Can you work these out from the model? Positions are in its coordinate system, mm. Face numbers are marked on the shaded views. A direction names the side the tool comes from. Give positions to 0.01 mm unless a question says otherwise; leave off trailing zeros. Order: outer loops, then holes, each group sorted by start corner. A loop starts at its lowest first (then second) coordinate and runs counter-clockwise, first axis right, second up. Notation, with made-up numbers: M 24.25,-38 L 63.25,-38 A21 cw 63.25,-20 Z; hole C 85.25,64 d8. An arc over 180 degrees is marked long. Use one line per item in the form item = value. Start each with the question number.
1. I need wall thicknesses on L1, parallel to Y at x = -41.5, z = 5.5; L2, parallel to X at y = 2, z = 3.25; L3, parallel to Y at x = -35, z = 1. Which ranges of each line are inside material? Lowest first, please.
2. For the marked faces 1 and 2, which set-ups out of +Z, -Z, +X, -X, +Y, -Y let a thin tool reach every point of the face, with its end or its side?
3. I want a section at B-B, the plane x = 44.5. List the corners of the cut face in (y, z) for me, and give its area (3 significant figures).
4. I want a section at D-D, the plane z = 4. Count the separate pieces of the cut face and the enclosed holes in it, and give its area (3 significant figures).
5. Will these pins go through, and if not, where does the flat tip stop? P1, Ø1.9, axis at x = 6.85, y = -23.16, coming from the -Z side; P2, Ø1, axis at x = 2, z = 8.5, coming from the +Y side.
6. I want a section at A-A, the plane y = 5.5. List the corners of the cut face in (x, z) for me, and give its area (3 significant figures).
7. I want a section at C-C, the plane y = 24. List the corners of the cut face in (x, z) for me.
8. We'd pull the mould along X, two halves only. Please class the marked faces 3, 4 and 5: +X half, -X half, draft (parallel to the pull), parting line (faces both ways), or undercut.
```python
from build123d import *

# Parameters (mm, degrees)
SKETCH_1_R      = 1.575
SKETCH_1_R_2    = 5
SKETCH_1_R_3    = 1.075
SKETCH_1_W      = 5
SKETCH_1_H      = 15
SKETCH_1_H_2    = 12.5
EXTRUDE_1_DEPTH = 12


with BuildPart() as part:
    # 草图1 → 凸台-拉伸1 (new body)
    with BuildSketch(Plane.XY):
        with BuildLine():
            Line((-33.144127259, 37.474667316), (-22.414010311, 15.474667316))
            Line((-22.414010311, 15.474667316), (22.585989689, 15.474667316))
            Line((22.585989689, 15.474667316), (33.316106638, 37.474667316))
            Line((33.316106638, 37.474667316), (47.885989689, 37.474667316))
            ThreePointArc((47.885989689, 37.474667316), (51.421523595, 36.010201222), (52.885989689, 32.474667316))
            Line((52.885989689, 32.474667316), (52.885989689, -32.525332684))
            ThreePointArc((52.885989689, -32.525332684), (51.421523595, -36.060866589), (47.885989689, -37.525332684))
            Line((47.885989689, -37.525332684), (-47.714010311, -37.525332684))
            ThreePointArc((-47.714010311, -37.525332684), (-51.249544217, -36.060866589), (-52.714010311, -32.525332684))
            Line((-52.714010311, -32.525332684), (-52.714010311, 32.474667316))
            ThreePointArc((-52.714010311, 32.474667316), (-51.249544217, 36.010201222), (-47.714010311, 37.474667316))
            Line((-47.714010311, 37.474667316), (-33.144127259, 37.474667316))
        make_face()
        with Locations((35.085989689, 31.055295289)):
            Circle(SKETCH_1_R, mode=Mode.SUBTRACT)
        with Locations((35.085989689, -31.444704711)):
            Circle(SKETCH_1_R, mode=Mode.SUBTRACT)
        with Locations((0.085989689, -11.444704711)):
            Circle(SKETCH_1_R_2, mode=Mode.SUBTRACT)
        with Locations((7.510989689, -11.444704711)):
            Circle(SKETCH_1_R_3, mode=Mode.SUBTRACT)
        with Locations((10.560989689, -11.444704711)):
            Circle(SKETCH_1_R_3, mode=Mode.SUBTRACT)
        with Locations((13.610989689, -11.444704711)):
            Circle(SKETCH_1_R_3, mode=Mode.SUBTRACT)
        with Locations((5.323489689, -20.516320815)):
            Circle(SKETCH_1_R_3, mode=Mode.SUBTRACT)
        with Locations((3.798489689, -17.874943334)):
            Circle(SKETCH_1_R_3, mode=Mode.SUBTRACT)
        with Locations((6.848489689, -23.157698297)):
            Circle(SKETCH_1_R_3, mode=Mode.SUBTRACT)
        with Locations((-5.151510311, -20.516320815)):
            Circle(SKETCH_1_R_3, mode=Mode.SUBTRACT)
        with Locations((-3.626510311, -17.874943334)):
            Circle(SKETCH_1_R_3, mode=Mode.SUBTRACT)
        with Locations((-6.676510311, -23.157698297)):
            Circle(SKETCH_1_R_3, mode=Mode.SUBTRACT)
        with Locations((-10.389010311, -11.444704711)):
            Circle(SKETCH_1_R_3, mode=Mode.SUBTRACT)
        with Locations((-7.339010311, -11.444704711)):
            Circle(SKETCH_1_R_3, mode=Mode.SUBTRACT)
        with Locations((-13.439010311, -11.444704711)):
            Circle(SKETCH_1_R_3, mode=Mode.SUBTRACT)
        with Locations((-5.151510311, -2.373088606)):
            Circle(SKETCH_1_R_3, mode=Mode.SUBTRACT)
        with Locations((-3.626510311, -5.014466088)):
            Circle(SKETCH_1_R_3, mode=Mode.SUBTRACT)
        with Locations((-6.676510311, 0.268288875)):
            Circle(SKETCH_1_R_3, mode=Mode.SUBTRACT)
        with Locations((5.323489689, -2.373088606)):
            Circle(SKETCH_1_R_3, mode=Mode.SUBTRACT)
        with Locations((3.798489689, -5.014466088)):
            Circle(SKETCH_1_R_3, mode=Mode.SUBTRACT)
        with Locations((6.848489689, 0.268288875)):
            Circle(SKETCH_1_R_3, mode=Mode.SUBTRACT)
        with Locations(Location((-34.914010311, 31.055295289, 0), (0, 0, 180))):
            Circle(SKETCH_1_R, mode=Mode.SUBTRACT)
        with Locations(Location((-34.914010311, -31.444704711, 0), (0, 0, 180))):
            Circle(SKETCH_1_R, mode=Mode.SUBTRACT)
        with Locations((-43.714010311, -23.525332684)):
            Rectangle(SKETCH_1_W, SKETCH_1_H, mode=Mode.SUBTRACT)
        with Locations((43.885989689, -23.525332684)):
            Rectangle(SKETCH_1_W, SKETCH_1_H, mode=Mode.SUBTRACT)
        with Locations((43.885989689, 1.474667316)):
            Rectangle(SKETCH_1_W, SKETCH_1_H_2, mode=Mode.SUBTRACT)
        with Locations((43.885989689, 26.474667316)):
            Rectangle(SKETCH_1_W, SKETCH_1_H, mode=Mode.SUBTRACT)
        with Locations((-43.714010311, 1.474667316)):
            Rectangle(SKETCH_1_W, SKETCH_1_H_2, mode=Mode.SUBTRACT)
        with Locations((-43.714010311, 26.474667316)):
            Rectangle(SKETCH_1_W, SKETCH_1_H, mode=Mode.SUBTRACT)
    extrude(amount=EXTRUDE_1_DEPTH)


solid = part.part
```
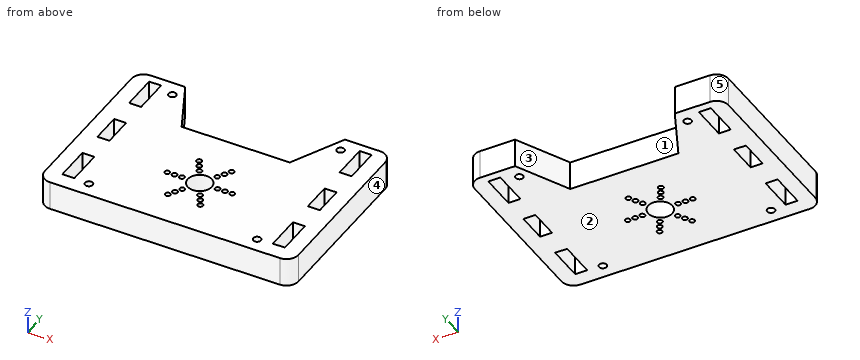
Check result:
q1.L1 = -37.53 to -31.03, -16.03 to -4.78, 7.72 to 18.97, 33.97 to 37.47
q1.L2 = -52.71 to -46.21, -41.21 to 41.39, 46.39 to 52.89
q1.L3 = -37.53 to -33.02, -29.87 to 29.48, 32.63 to 37.47
q2.face_1 = +Z, -Z, +Y
q2.face_2 = -Z, +X, -X, +Y, -Y
q3.outline = M -37.53,0 L -31.03,0 L -31.03,12 L -37.53,12 Z; M -16.03,0 L -4.78,0 L -4.78,12 L -16.03,12 Z; M 7.72,0 L 18.97,0 L 18.97,12 L 7.72,12 Z; M 33.97,0 L 37.47,0 L 37.47,12 L 33.97,12 Z
q3.area = 390 mm2
q4.separate_pieces = 1
q4.enclosed_holes = 29
q4.area = 6,070 mm2
q5.P1 = through
q5.P2 = 15.47
q6.outline = M -52.71,0 L -46.21,0 L -46.21,12 L -52.71,12 Z; M -41.21,0 L 41.39,0 L 41.39,12 L -41.21,12 Z; M 46.39,0 L 52.89,0 L 52.89,12 L 46.39,12 Z
q6.area = 1,150 mm2
q7.outline = M -52.71,0 L -46.21,0 L -46.21,12 L -52.71,12 Z; M -41.21,0 L -26.57,0 L -26.57,12 L -41.21,12 Z; M 26.74,0 L 41.39,0 L 41.39,12 L 26.74,12 Z; M 46.39,0 L 52.89,0 L 52.89,12 L 46.39,12 Z
q8.face_3 = undercut
q8.face_4 = +X half
q8.face_5 = -X half
